Build history of the part. All positions in model axes, mm. Face numbers are marked on the shaded views. Give positions to 0.01 mm unless a question says otherwise; leave off trailing zeros. Write each loop counter-clockwise with the first axis right and the second up, starting at its lowest first coordinate (ties: lowest second). Pieces come first, ordered by that corner, then holes. Notation, with made-up numbers: M 40,-16 L 81,-16 A28 ccw 81,14 Z; hole C 2,16 d4. An arc over 180 degrees is marked long. One line per item, written item: value. Start each with the question number.
from build123d import *

# Parameters (mm, degrees)
SKETCH1_W           = 50
SKETCH1_H           = 45
SKETCH1_R           = 9
BOSS_EXTRUDE1_DEPTH = 20
FILLET1_R           = 10


with BuildPart() as part:
    # Sketch1 → Boss-Extrude1 (new body)
    with BuildSketch(Plane.XY):
        with Locations((25, 22.5)):
            Rectangle(SKETCH1_W, SKETCH1_H)
        with Locations((25, 30)):
            Circle(SKETCH1_R, mode=Mode.SUBTRACT)
    extrude(amount=BOSS_EXTRUDE1_DEPTH)

    # Fillet1
    fillet1_edges = [part.edges().sort_by_distance(p)[0] for p in [
        (0, 45, 10),
        (50, 45, 10),
    ]]
    fillet(fillet1_edges, radius=FILLET1_R)


solid = part.part
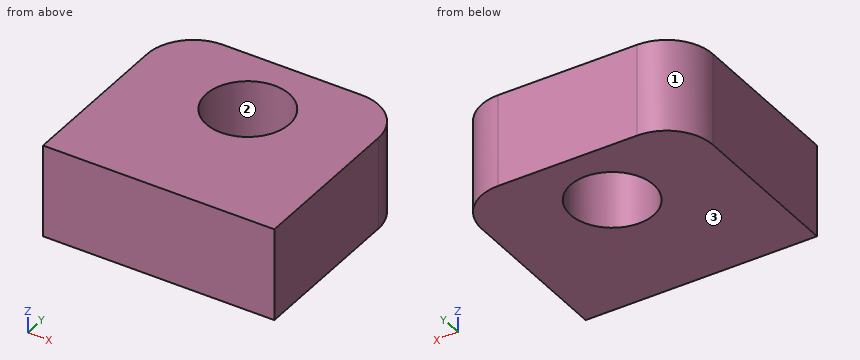
1) Probe line 1 along Y through (x, z) = (25, 6.5); line 2 along X through (y, z) = (29, 6); line 3 along Y through (x, z) = (27, 5.75). List the from-to ranges inside material, lowest first. Write a range as from..to.
2) Mould opens along Y. For the marked faces 1, 2 and 3 say: released by +Y, released by -Y, zero draft, split by the parting line, or undercut.
3) Band-saw the part on C-C (y = 30). List the corners of the cut face in (x, z), then the cut area to 3 significant figures.
4) Band-saw the part on B-B (z = 6). List the corners of the cut face in (x, y), then the cut area to 3 significant figures.
5) Drop a flat-ended pin along its axis: P1, Ø1, axis at y = 40.5, z = 3.5, coming from the -X side. Give the stop position or say it passes through.
6) Band-saw the part on D-D (x = 45.5). List the corners of the cut face in (y, z).
7) Band-saw the part on A-A (x = 25). List the corners of the cut face in (y, z), then the cut area to 3 significant figures.
Model answer:
1. line 1: y = 0..21, 39..45
1. line 2: x = 0..16.06, 33.94..50
1. line 3: y = 0..21.23, 38.77..45
2. face 1: released by +Y
2. face 2: undercut
2. face 3: zero draft
3. outline: M 0,0 L 16,0 L 16,20 L 0,20 Z; M 34,0 L 50,0 L 50,20 L 34,20 Z
3. area: 640 mm²
4. outline: M 0,0 L 50,0 L 50,35 A10 ccw 40,45 L 10,45 A10 ccw 0,35 Z; hole C 25,30 d18
4. area: 1,950 mm²
5. P1: stops at x = 1.34
6. outline: M 0,0 L 43.35,0 L 43.35,20 L 0,20 Z
7. outline: M 0,0 L 21,0 L 21,20 L 0,20 Z; M 39,0 L 45,0 L 45,20 L 39,20 Z
7. area: 540 mm²
